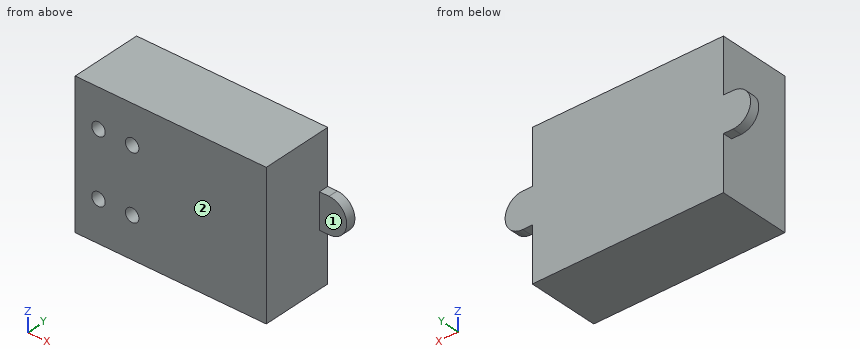
```python
from build123d import *

# Parameters (mm, degrees)
SKETCH1_W           = 40
SKETCH1_H           = 30
BOSS_EXTRUDE1_DEPTH = 15
BOSS_EXTRUDE2_DEPTH = 2
SKETCH3_R           = 1.408779943
CUT_EXTRUDE1_DEPTH  = 5


with BuildPart() as part:
    # Sketch1 → Boss-Extrude1 (new body)
    with BuildSketch(Plane(origin=(0, 0, 0), x_dir=(1, 0, 0), z_dir=(0, 1, 0))):
        Rectangle(SKETCH1_W, SKETCH1_H)
    extrude(amount=BOSS_EXTRUDE1_DEPTH)

    # Sketch2 → Boss-Extrude2 (add)
    with BuildSketch(Plane(origin=(0, 15, 0), x_dir=(1, 0, 0), z_dir=(0, 1, 0))):
        with BuildLine():
            Line((-21.995796848, 3.691602268), (21.995796848, 3.691602268))
            ThreePointArc((21.995796848, 3.691602268), (25.687399116, 0), (21.995796848, -3.691602268))
            Line((21.995796848, -3.691602268), (-21.995796848, -3.691602268))
            ThreePointArc((-21.995796848, -3.691602268), (-25.687399116, 0), (-21.995796848, 3.691602268))
        make_face()
    extrude(amount=-BOSS_EXTRUDE2_DEPTH)

    # Sketch3 → Cut-Extrude1 (cut)
    with BuildSketch(Plane.XZ):
        with Locations(Location((-15.114073065, 6.951101682, 0), (0, 0, 270))):
            Circle(SKETCH3_R)
        with Locations(Location((-8.071509519, 6.951101682, 0), (0, 0, 270))):
            Circle(SKETCH3_R)
        with Locations(Location((-15.114073065, -6.448061429, 0), (0, 0, 270))):
            Circle(SKETCH3_R)
        with Locations(Location((-8.071509519, -6.448061429, 0), (0, 0, 270))):
            Circle(SKETCH3_R)
    extrude(amount=-CUT_EXTRUDE1_DEPTH, mode=Mode.SUBTRACT)


solid = part.part
```
Input: part model. Units: mm. Frame: model coordinates. Face numbers are marked on the shaded views. A direction names the side the tool comes from. Round coordinates to 2 decimals unless told otherwise and drop trailing zeros. Loops run counter-clockwise (first coordinate to the right, second up) from the corner with the lowest first, then second, coordinate; pieces in that order, holes last. Notation, with made-up numbers: (-8.75, 44.5) - (48.25, 44.5) arc R7 ccw to (48.25, 50.5) - close; hole circle Ø8 at (87, 4.25). An arc over 180 degrees is marked (long way). One line per item, written item: value. Start each with the question number.
(1) Ray query, line 1 (X direction, y = 2.5, z = 7); line 2 (Z direction, x = -7, y = 2); line 3 (X direction, y = 2.25, z = 6.25). Return the intervals inside material, ascending. Write a range as [from, to].
(2) Section B-B, the plane x = -16. Return loops of the section in (y, z).
(3) Access query for the marked faces 1 and 2. Directions: +Z, -Z, +X, -X, +Y, -Y. A direction counts if a zero-diameter tool reaches every point of the face in a straight line with its end or side. Return the directions, or none.
(4) Section D-D, the plane z = -6.25. Return loops of the section in (x, y).
(5) Contact query for flat-ended pins moving along their axis: P1, Ø1.5, axis at x = 0, z = -9.5, coming from the -Y side; P2, Ø1.4, axis at x = -15.5, z = -6.5, coming from the -Y side; P3, Ø7.5, axis at y = 9, z = 2.5, coming from the +X side; P4, Ø2, axis at x = -21.5, y = 14, coming from the -Z side. Output: stop coordinate, or through.
(6) Section A-A, the plane z = 0. Return loops of the section in (x, y), plus the area to 3 significant figures.
(7) Section C-C, the plane y = 9.75. Return loops of the section in (x, z).
Results below:
1. line 1: [-20, -16.52], [-13.71, -9.48], [-6.66, 20]
1. line 2: [-15, -7.36], [-5.53, 6.04], [7.87, 15]
1. line 3: [-20, -16.34], [-13.89, -9.29], [-6.85, 20]
2. outline: (0, -15) - (15, -15) - (15, 15) - (0, 15) - (0, 8.05) - (5, 8.05) - (5, 5.86) - (0, 5.86) - (0, -5.35) - (5, -5.35) - (5, -7.54) - (0, -7.54) - close
3. face 1: +Z, -Z, +X, -Y
3. face 2: +Z, -Z, +X, -X, -Y
4. outline: (-20, 0) - (-16.51, 0) - (-16.51, 5) - (-13.72, 5) - (-13.72, 0) - (-9.47, 0) - (-9.47, 5) - (-6.68, 5) - (-6.68, 0) - (20, 0) - (20, 15) - (-20, 15) - close
5. P1: y = 0
5. P2: y = 5
5. P3: x = 20
5. P4: z = -3.69
6. outline: (-25.69, 13) - (-20, 13) - (-20, 0) - (20, 0) - (20, 13) - (25.69, 13) - (25.69, 15) - (-25.69, 15) - close
6. area: 623 mm^2
7. outline: (-20, -15) - (20, -15) - (20, 15) - (-20, 15) - close
